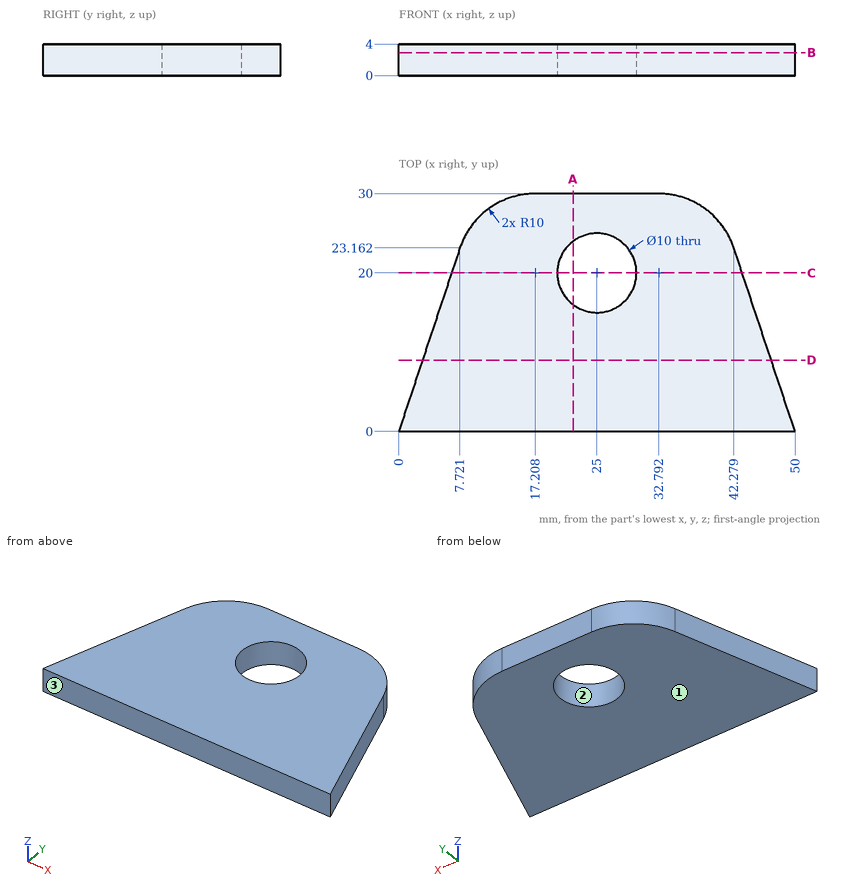
Answer from the drawing. Dimensions are ordinates in mm from the lowest x, y and z of the part. Coordinates: 2 decimals unless noted, no trailing zeros. Order: outer loops, then holes, each group sorted by start corner. A loop starts at its lowest first (then second) coordinate and runs counter-clockwise, first axis right, second up. Notation, with made-up numbers: M -28,37 L -14,37 A8 ccw -14,50 Z; hole C -17,50.5 d8. An arc over 180 degrees is marked long. Put each result on its own line as item: value. Start each with the question number.
Item 1: The mould has two halves that part along Y. Classify the marked faces 1, 2 and 3: +Y half, -Y half, draft (parallel to the pull), parting line (faces both ways), or undercut.
Item 2: Section C-C, the plane y = 20 is taken. Determine the outline of the cut face in (x, z), plus the area to 3 significant figures.
Item 3: Consider probe 1 along Y at (x, z) = (25, 1.8); probe 2 along Y at (x, z) = (22, 1.2); probe 3 along X at (y, z) = (16, 2.95) (1 decimal). Determine where each line is inside the solid, lowest interval first. Write a range as [from, to].
Item 4: Section D-D, the plane y = 9 is taken. Determine the outline of the cut face in (x, z).
Item 5: Given pin 1 Ø12 at (x, y) = (24, 24.5) entering from +Z; pin 2 Ø2 at (x, z) = (37.5, 3) entering from +Y, each flat-ended and moving along its own axis, determine where each tip first touches the part or whether it passes through.
Item 6: Section B-B, the plane z = 2.9 is taken. Determine the outline of the cut face in (x, y).
Item 7: Section A-A, the plane x = 22 is taken. Determine the outline of the cut face in (y, z).
Computed:
1. face 1: draft
1. face 2: undercut
1. face 3: -Y half
2. outline: M 6.67,0 L 20,0 L 20,4 L 6.67,4 Z; M 30,0 L 43.33,0 L 43.33,4 L 30,4 Z
2. area: 107 mm2
3. probe 1: y = [0, 15], [25, 30]
3. probe 2: y = [0, 16], [24, 30]
3. probe 3: x = [5.3, 22], [28, 44.7]
4. outline: M 3,0 L 47,0 L 47,4 L 3,4 Z
5. pin 1: stops at z = 4
5. pin 2: stops at y = 29.29
6. outline: M 0,0 L 50,0 L 42.28,23.16 A10 ccw 32.79,30 L 17.21,30 A10 ccw 7.72,23.16 Z; hole C 25,20 d10
7. outline: M 0,0 L 16,0 L 16,4 L 0,4 Z; M 24,0 L 30,0 L 30,4 L 24,4 Z
